```python
from build123d import *

# Parameters (mm, degrees)
SKETCH1_W               = 200
SKETCH1_H               = 200
BOSS_EXTRUDE1_DEPTH     = 15
SKETCH2_R               = 4
CUT_EXTRUDE1_DEPTH      = 25
LPATTERN1_COUNT         = 2
LPATTERN1_PITCH         = 75
MIRROR1_COPY_1_SKETCH_R = 4
MIRROR1_COPY_1_DEPTH    = 25
MIRROR2_COPY_1_SKETCH_R = 4
MIRROR2_COPY_1_DEPTH    = 25
MIRROR2_COPY_2_SKETCH_R = 4
MIRROR2_COPY_2_DEPTH    = 25
MIRROR2_COPY_3_SKETCH_R = 4
MIRROR2_COPY_3_DEPTH    = 25
SKETCH3_R               = 4
CUT_EXTRUDE2_DEPTH      = 25
LPATTERN2_COUNT         = 2
LPATTERN2_PITCH         = 85
MIRROR3_COPY_1_SKETCH_R = 4
MIRROR3_COPY_1_DEPTH    = 25
MIRROR4_COPY_1_SKETCH_R = 4
MIRROR4_COPY_1_DEPTH    = 25
MIRROR4_COPY_2_SKETCH_R = 4
MIRROR4_COPY_2_DEPTH    = 25
MIRROR4_COPY_3_SKETCH_R = 4
MIRROR4_COPY_3_DEPTH    = 25


with BuildPart() as part:
    # Sketch1 → Boss-Extrude1 (new body)
    with BuildSketch(Plane.XY):
        Rectangle(SKETCH1_W, SKETCH1_H)
    extrude(amount=BOSS_EXTRUDE1_DEPTH)

    # Sketch2 → Cut-Extrude1 (cut)
    with BuildSketch(Plane(origin=(100, 0, 0), x_dir=(0, 0, -1), z_dir=(1, 0, 0))):
        with Locations((-7.5, 0)):
            Circle(SKETCH2_R)
    cut_extrude1 = extrude(amount=-CUT_EXTRUDE1_DEPTH, mode=Mode.SUBTRACT)

    # LPattern1: Cut-Extrude1 ×2
    with Locations(*[(0, -i * LPATTERN1_PITCH, 0) for i in range(1, LPATTERN1_COUNT)]):
        add(cut_extrude1, mode=Mode.SUBTRACT)

    # Mirror1: Cut-Extrude1 across plane
    add(cut_extrude1.mirror(Plane.ZX), mode=Mode.SUBTRACT)

    # Mirror1 copy 1 sketch → Mirror1 copy 1 (cut)
    with BuildSketch(Plane(origin=(100, 75, 0), x_dir=(0, 0, -1), z_dir=(1, 0, 0))):
        with Locations((-7.5, 0)):
            Circle(MIRROR1_COPY_1_SKETCH_R)
    extrude(amount=-MIRROR1_COPY_1_DEPTH, mode=Mode.SUBTRACT)

    # Mirror2: Cut-Extrude1 across plane
    add(cut_extrude1.mirror(Plane(origin=(0, 0, 0), x_dir=(0, 0, 1), z_dir=(1, 0, 0))), mode=Mode.SUBTRACT)

    # Mirror2 copy 1 sketch → Mirror2 copy 1 (cut)
    with BuildSketch(Plane(origin=(-100, -75, 0), x_dir=(0, 0, -1), z_dir=(-1, 0, 0))):
        with Locations((-7.5, 0)):
            Circle(MIRROR2_COPY_1_SKETCH_R)
    extrude(amount=-MIRROR2_COPY_1_DEPTH, mode=Mode.SUBTRACT)

    # Mirror2 copy 2 sketch → Mirror2 copy 2 (cut)
    with BuildSketch(Plane(origin=(-100, 0, 0), x_dir=(0, 0, -1), z_dir=(-1, 0, 0))):
        with Locations((-7.5, 0)):
            Circle(MIRROR2_COPY_2_SKETCH_R)
    extrude(amount=-MIRROR2_COPY_2_DEPTH, mode=Mode.SUBTRACT)

    # Mirror2 copy 3 sketch → Mirror2 copy 3 (cut)
    with BuildSketch(Plane(origin=(-100, 75, 0), x_dir=(0, 0, -1), z_dir=(-1, 0, 0))):
        with Locations((-7.5, 0)):
            Circle(MIRROR2_COPY_3_SKETCH_R)
    extrude(amount=-MIRROR2_COPY_3_DEPTH, mode=Mode.SUBTRACT)

    # Sketch3 → Cut-Extrude2 (cut)
    with BuildSketch(Plane(origin=(0, 100, 0), x_dir=(1, 0, 0), z_dir=(0, 1, 0))):
        with Locations(Location((0, -7.5, 0), (0, 0, 180))):
            Circle(SKETCH3_R)
    cut_extrude2 = extrude(amount=-CUT_EXTRUDE2_DEPTH, mode=Mode.SUBTRACT)

    # LPattern2: Cut-Extrude2 ×2
    with Locations(*[(i * LPATTERN2_PITCH, 0, 0) for i in range(1, LPATTERN2_COUNT)]):
        add(cut_extrude2, mode=Mode.SUBTRACT)

    # Mirror3: Cut-Extrude2 across plane
    add(cut_extrude2.mirror(Plane(origin=(0, 0, 0), x_dir=(0, 0, 1), z_dir=(1, 0, 0))), mode=Mode.SUBTRACT)

    # Mirror3 copy 1 sketch → Mirror3 copy 1 (cut)
    with BuildSketch(Plane(origin=(-85, 100, 0), x_dir=(-1, 0, 0), z_dir=(0, 1, 0))):
        with Locations((0, 7.5)):
            Circle(MIRROR3_COPY_1_SKETCH_R)
    extrude(amount=-MIRROR3_COPY_1_DEPTH, mode=Mode.SUBTRACT)

    # Mirror4: Cut-Extrude2 across plane
    add(cut_extrude2.mirror(Plane.ZX), mode=Mode.SUBTRACT)

    # Mirror4 copy 1 sketch → Mirror4 copy 1 (cut)
    with BuildSketch(Plane(origin=(85, -100, 0), x_dir=(1, 0, 0), z_dir=(0, -1, 0))):
        with Locations((0, 7.5)):
            Circle(MIRROR4_COPY_1_SKETCH_R)
    extrude(amount=-MIRROR4_COPY_1_DEPTH, mode=Mode.SUBTRACT)

    # Mirror4 copy 2 sketch → Mirror4 copy 2 (cut)
    with BuildSketch(Plane(origin=(0, -100, 0), x_dir=(-1, 0, 0), z_dir=(0, -1, 0))):
        with Locations(Location((0, -7.5, 0), (0, 0, 180))):
            Circle(MIRROR4_COPY_2_SKETCH_R)
    extrude(amount=-MIRROR4_COPY_2_DEPTH, mode=Mode.SUBTRACT)

    # Mirror4 copy 3 sketch → Mirror4 copy 3 (cut)
    with BuildSketch(Plane(origin=(-85, -100, 0), x_dir=(-1, 0, 0), z_dir=(0, -1, 0))):
        with Locations(Location((0, -7.5, 0), (0, 0, 180))):
            Circle(MIRROR4_COPY_3_SKETCH_R)
    extrude(amount=-MIRROR4_COPY_3_DEPTH, mode=Mode.SUBTRACT)


solid = part.part
```
Geometry: final body of the model. Coordinates: model frame, mm. A direction names the side the tool comes from. Round coordinates to 2 decimals unless told otherwise and drop trailing zeros. Write each loop counter-clockwise with the first axis right and the second up, starting at its lowest first coordinate (ties: lowest second). Pieces come first, ordered by that corner, then holes.
Item 1: Mould query, pull axis X, two halves, no side actions, for faces 4 (the face through (-81.004, 87.675, 7.676)), 5 (the face through (-75, 75, 8)), 6 (the face through (0, 75, 8)), 7 (the face through (-1, -100, 12)). Classes: +X half, -X half, draft (parallel to the pull), parting line (faces both ways), or undercut.
Item 2: Material intervals for L1, parallel to X at y = 92.5, z = 7.5; L2, parallel to Y at x = 95, z = 7.5; L3, parallel to Z at x = -85, y = -89, sorted ascending.
Item 3: Section query B-B (x = 85). Return loops of the section in (y, z), plus the area to 3 significant figures.
Item 4: Section query C-C (x = 0). Return loops of the section in (y, z), plus the area to 3 significant figures.
Item 5: Pin query (flat end, axial travel): P1, Ø6.5, axis at x = -85, z = 7.5, coming from the -Y side; P2, Ø5, axis at y = 0, z = 7.5, coming from the +X side; P3, Ø4, axis at y = -76, z = 7, coming from the -X side. Return the tip coordinate at first contact, or that it passes through.
Item 6: Set-up query: faces 1 (the face through (81.004, -87.675, 7.676)), 2 (the face through (88.996, 87.675, 7.676)), 3 (the face through (75, 75, 8)). Return all of +Z, -Z, +X, -X, +Y, -Y with unobstructed straight access to the full face (end or side cutting, diameter ignored); none if empty.
Item 7: Section query A-A (x = -77.5). Return loops of the section in (y, z).
Completed:
1. face 4: undercut
1. face 5: -X half
1. face 6: undercut
1. face 7: draft
2. L1: x = -100 to -89, -81 to -4, 4 to 81, 89 to 100
2. L2: y = -100 to -79, -71 to -4, 4 to 71, 79 to 100
2. L3: z = 0 to 3.5, 11.5 to 15
3. outline: (-100, 0) - (100, 0) - (100, 3.5) - (75, 3.5) arc R4 cw to (75, 11.5) - (100, 11.5) - (100, 15) - (-100, 15) - (-100, 11.5) - (-75, 11.5) arc R4 cw to (-75, 3.5) - (-100, 3.5) - close; hole circle Ø8 at (0, 7.5)
3. area: 2,500 mm2
4. outline: (-100, 0) - (100, 0) - (100, 3.5) - (75, 3.5) - (75, 11.5) - (100, 11.5) - (100, 15) - (-100, 15) - (-100, 11.5) - (-75, 11.5) - (-75, 3.5) - (-100, 3.5) - close
4. area: 2,600 mm2
5. P1: stops at y = -72.67
5. P2: stops at x = 75
5. P3: stops at x = -75
6. face 1: -Y
6. face 2: +Y
6. face 3: +X
7. outline: (-100, 0) - (100, 0) - (100, 15) - (-100, 15) - close; hole circle Ø8 at (-75, 7.5); hole circle Ø8 at (0, 7.5); hole circle Ø8 at (75, 7.5)
